Check sheet for the drawn part. Datum: minimum x, y, z corner. Units: mm. A direction names the side the tool comes from. Give positions to 0.01 mm unless a question says otherwise; leave off trailing zeros. Write each loop counter-clockwise with the first axis right and the second up, starting at its lowest first coordinate (ties: lowest second). Pieces come first, ordered by that corner, then holes. Notation, with made-up numbers: M 8,45.5 L 62,45.5 A20 cw 62,79.5 Z; hole C 69.25,80.5 d3. An arc over 180 degrees is marked long. Write item = value, one per line. Start each with the question number.
1) Set-up check for the marked faces 4 and 5: record each of +Z, -Z, +X, -X, +Y, -Y from which the full face is reachable in a straight line by a thin tool's end or side.
2) Gauge pin test, flat end, axial feed: pin 1 (4 mm diameter, centred on x = 6, z = 10, fed in from +Y). Record the tip position at first contact, or that the pin passes through.
3) Sectioned sample at D-D, the plane y = 10. Record the cut outline in (x, z).
4) Sectioned sample at A-A, the plane z = 10. Record the cut outline in (x, y).
5) Scan lines: L1, parallel to Z at x = 61.5, y = 12.25; L2, parallel to X at y = 4.5, z = 10. Record each from-to range of solid material in increasing order.
6) Sectioned sample at C-C, the plane z = 2.25. Record the cut outline in (x, y), then the cut area to 3 significant figures.
7) Draft check along X on the marked faces 1, 2 and 3. Enter one of: pulls with the +X half, pulls with the -X half, needs draft (parallel to the pull), parting line crosses it, or undercut.
8) Sectioned sample at B-B, the plane x = 6. Record the cut outline in (y, z), then the cut area to 3 significant figures.
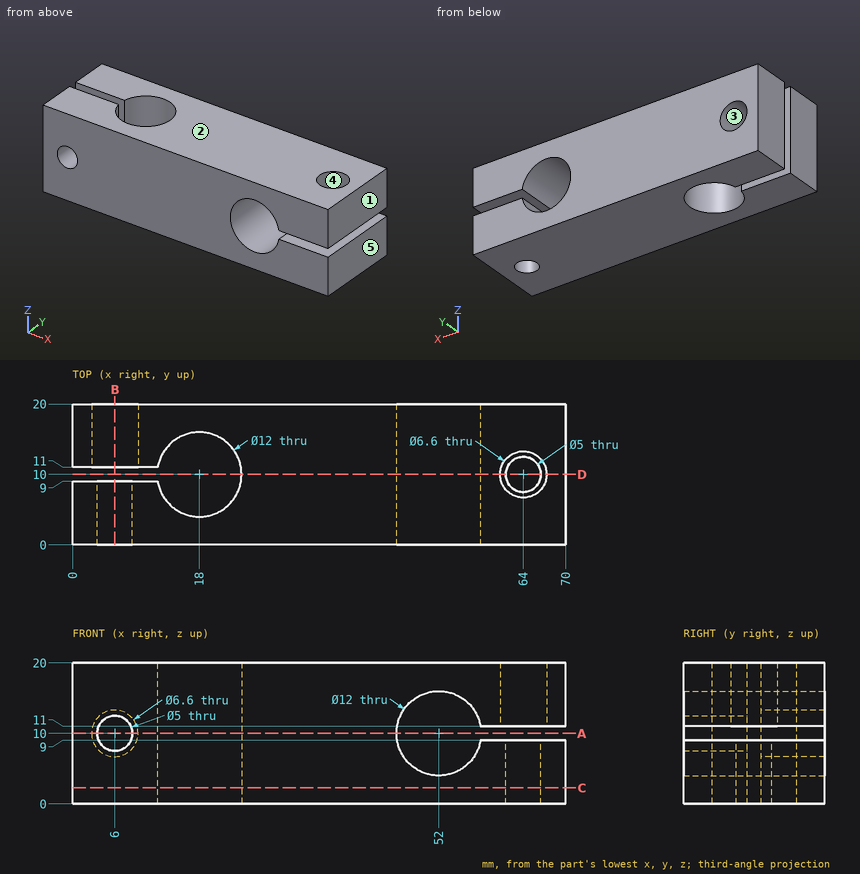
Data:
q1.face_4 = +Z
q1.face_5 = +Z, -Z, +X, +Y, -Y
q2.pin_1 = through
q3.outline = M 24,0 L 61.5,0 L 61.5,9 L 57.92,9 A6 cw long 57.92,11 L 60.7,11 L 60.7,20 L 24,20 Z; M 66.5,0 L 70,0 L 70,9 L 66.5,9 Z; M 67.3,11 L 70,11 L 70,20 L 67.3,20 Z
q4.outline = M 0,0 L 3.5,0 L 3.5,9 L 0,9 Z; M 0,11 L 2.7,11 L 2.7,20 L 0,20 Z; M 8.5,0 L 46,0 L 46,20 L 9.3,20 L 9.3,11 L 12.08,11 A6 cw long 12.08,9 L 8.5,9 Z
q5.L1 = 0 to 9, 11 to 20
q5.L2 = 0 to 3.5, 8.5 to 15.6, 20.4 to 46
q6.outline = M 0,0 L 70,0 L 70,20 L 0,20 L 0,11 L 12.08,11 A6 cw long 12.08,9 L 0,9 Z; hole C 64,10 d5
q6.area = 1,240 mm2
q7.face_1 = pulls with the +X half
q7.face_2 = needs draft
q7.face_3 = undercut
q8.outline = M 0,0 L 9,0 L 9,7.5 L 0,7.5 Z; M 0,12.5 L 9,12.5 L 9,20 L 0,20 Z; M 11,0 L 20,0 L 20,6.7 L 11,6.7 Z; M 11,13.3 L 20,13.3 L 20,20 L 11,20 Z
q8.area = 256 mm2
